```python
from build123d import *

# Parameters (mm, degrees)
SKETCH_3_R      = 28
SKETCH_3_R_2    = 23
EXTRUDE_1_DEPTH = 90
SKETCH_4_R      = 23.5
SKETCH_4_R_2    = 11
EXTRUDE_2_DEPTH = 4
CHAMFER_1_SIZE  = 0.2


with BuildPart() as part:
    # 草图3 → 凸台-拉伸1 (new body)
    with BuildSketch(Plane(origin=(0, 0, 0), x_dir=(1, 0, 0), z_dir=(0, 1, 0))):
        with Locations(Location((0, 0, 0), (0, 0, 90))):
            Circle(SKETCH_3_R)
        with Locations(Location((0, 0, 0), (0, 0, 90))):
            Circle(SKETCH_3_R_2, mode=Mode.SUBTRACT)
    extrude(amount=EXTRUDE_1_DEPTH)

    # 草图4 → 凸台-拉伸2 (add)
    with BuildSketch(Plane.XZ.offset(-90)):
        Circle(SKETCH_4_R)
        with Locations(Location((0, 0, 0), (0, 0, 270))):
            Circle(SKETCH_4_R_2, mode=Mode.SUBTRACT)
    extrude(amount=EXTRUDE_2_DEPTH)

    # 倒角1
    chamfer_1_edges = [part.edges().sort_by_distance(p)[0] for p in [
        (0, 90, 11),
        (0, 0, 28),
        (0, 90, 28),
        (0, 0, 23),
    ]]
    chamfer(chamfer_1_edges, length=CHAMFER_1_SIZE)


solid = part.part
```
The listing builds one solid part. Answer for the finished solid, in the listing's coordinates (mm). A direction names the side the tool comes from. Give positions to 0.01 mm unless a question says otherwise; leave off trailing zeros. Order: outer loops, then holes, each group sorted by start corner. A loop starts at its lowest first (then second) coordinate and runs counter-clockwise, first axis right, second up. Notation, with made-up numbers: M 4.5,-14 L 62.5,-14 A26 cw 62.5,7 Z; hole C 80.25,18 d8. An arc over 180 degrees is marked long. Put each result on its own line as item: value. Start each with the question number.
Item 1: Which of the six approach directions +Z, -Z, +X, -X, +Y, -Y give full straight-line access (tool end or side, diameter ignored) to faces 1 (the face through (12, 90, 0)), 2 (the face through (10, 86, 5))?
Item 2: Find the intervals of material crossed by line 1 along Z through (x, y) = (-1, 25); line 2 along X through (y, z) = (88.2, 0); line 3 along X through (y, z) = (11, -0.5), in increasing order.
Item 3: For a pull along Z with two mould halves and no side action, classify faces 3 (the face through (27.334, 44.373, 6.07)), 4 (the face through (23, 0, 6)), 5 (the face through (-10.74, 87.93, 2.38)) as +Z half, -Z half, draft (parallel to the pull), parting line (faces both ways), or undercut.
Item 4: The part is cut by section B-B, the plane z = 0. Determine the outline of the cut face in (x, y), and give its area (3 significant figures).
Item 5: The part is cut by section A-A, the plane x = 0. Determine the outline of the cut face in (y, z), and give its area (3 significant figures).
Item 6: Flat-ended cylindrical pins translate along their axes: P1, Ø8, axis at x = 11, z = 9, coming from the -Y side; P2, Ø1.5, axis at x = -16.5, y = 27.5, coming from the +Z side; P3, Ø8, axis at y = 79, z = -17.5, coming from the -X side. Find the tip coordinate at first contact, or state that the pin passes through.
Item 7: The part is cut by section C-C, the plane y = 9.5. Determine the outline of the cut face in (x, z).
Answer key:
1. face 1: +Z, -Z, +X, -X, +Y
1. face 2: -Y
2. line 1: z = -27.98 to -22.98, 22.98 to 27.98
2. line 2: x = -28 to -11, 11 to 28
2. line 3: x = -28 to -22.99, 22.99 to 28
3. face 3: parting line
3. face 4: draft
3. face 5: undercut
4. outline: M -28,0.2 L -27.8,0 L -23.2,0 L -23,0.2 L -23,86 L -11,86 L -11,89.8 L -11.2,90 L -27.8,90 L -28,89.8 Z; M 11,86 L 23,86 L 23,0.2 L 23.2,0 L 27.8,0 L 28,0.2 L 28,89.8 L 27.8,90 L 11.2,90 L 11,89.8 Z
4. area: 996 mm²
5. outline: M 0,-27.8 L 0.2,-28 L 89.8,-28 L 90,-27.8 L 90,-11.2 L 89.8,-11 L 86,-11 L 86,-23 L 0.2,-23 L 0,-23.2 Z; M 0,23.2 L 0.2,23 L 86,23 L 86,11 L 89.8,11 L 90,11.2 L 90,27.8 L 89.8,28 L 0.2,28 L 0,27.8 Z
5. area: 996 mm²
6. P1: stops at y = 86
6. P2: stops at z = 23.15
6. P3: stops at x = -24.53
7. outline: C 0,0 d56; hole C 0,0 d46
